Can you work these out from the model? Positions are in its coordinate system, mm. Face numbers are marked on the shaded views. A direction names the side the tool comes from. Coordinates: 2 decimals unless noted, no trailing zeros. Order: outer loops, then holes, each group sorted by start corner. A loop starts at its lowest first (then second) coordinate and runs counter-clockwise, first axis right, second up.
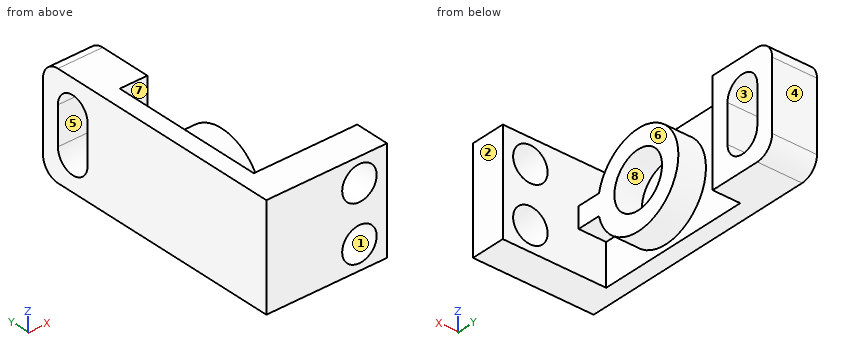
```python
from build123d import *

# Parameters (mm, degrees)
BASE_PLATE_SKETCH_W     = 35
BASE_PLATE_SKETCH_H     = 10
BASE_PLATE_DEPTH        = 30
UPRIGHT_WALL_SKETCH_W   = 5
UPRIGHT_WALL_SKETCH_H   = 45
UPRIGHT_WALL_DEPTH      = 30
MOUNTING_HOLES_SKETCH_R = 5
MOUNTING_HOLES_2X_DEPTH = 30
TOP_LUG_DEPTH           = 8
TOP_LUG_DEPTH_BACK      = 5
LUG_SLOT_DEPTH          = 84.719770664
RING_BOSS_SKETCH_R      = 8
RING_BOSS_DEPTH         = 8


with BuildPart() as part:
    # Base Plate Sketch → Base Plate (new body)
    with BuildSketch(Plane.XY):
        with Locations((17.5, 5)):
            Rectangle(BASE_PLATE_SKETCH_W, BASE_PLATE_SKETCH_H)
    extrude(amount=-BASE_PLATE_DEPTH)

    # Upright Wall Sketch → Upright Wall (add)
    with BuildSketch(Plane.XY):
        with Locations((2.5, 32.5)):
            Rectangle(UPRIGHT_WALL_SKETCH_W, UPRIGHT_WALL_SKETCH_H)
    extrude(amount=-UPRIGHT_WALL_DEPTH)

    # Mounting Holes Sketch → Mounting Holes 2x (cut)
    with BuildSketch(Plane(origin=(0, 10, 0), x_dir=(1, 0, 0), z_dir=(0, 1, 0))):
        with Locations(Location((27, 23, 0), (0, 0, 270))):
            Circle(MOUNTING_HOLES_SKETCH_R)
        with Locations(Location((27, 7, 0), (0, 0, 270))):
            Circle(MOUNTING_HOLES_SKETCH_R)
    extrude(amount=-MOUNTING_HOLES_2X_DEPTH, mode=Mode.SUBTRACT)

    # Top Lug Sketch → Top Lug (add, two sides: drawn at the far end of the back side and taken through both)
    with BuildSketch(Plane(origin=(5, 0, 0), x_dir=(0, 0, -1), z_dir=(1, 0, 0)).offset(-TOP_LUG_DEPTH_BACK)):
        with BuildLine():
            Line((0, 55), (30, 55))
            Line((30, 55), (30, 70))
            ThreePointArc((30, 70), (28.535533906, 73.535533906), (25, 75))
            Line((25, 75), (5, 75))
            ThreePointArc((5, 75), (1.464466094, 73.535533906), (0, 70))
            Line((0, 70), (0, 55))
        make_face()
    extrude(amount=TOP_LUG_DEPTH + TOP_LUG_DEPTH_BACK)

    # Lug Slot Sketch → Lug Slot (cut, through all)
    with BuildSketch(Plane(origin=(13, 0, 0), x_dir=(0, 0, -1), z_dir=(1, 0, 0))):
        with BuildLine():
            Line((9.5, 70), (20.5, 70))
            ThreePointArc((20.5, 70), (25.5, 65), (20.5, 60))
            Line((20.5, 60), (9.5, 60))
            ThreePointArc((9.5, 60), (4.5, 65), (9.5, 70))
        make_face()
    extrude(amount=-LUG_SLOT_DEPTH, mode=Mode.SUBTRACT)

    # Ring Boss Sketch → Ring Boss (add)
    with BuildSketch(Plane(origin=(5, 0, 0), x_dir=(0, 0, -1), z_dir=(1, 0, 0))):
        with BuildLine():
            Line((12, 16.837553419), (12, 10))
            Line((12, 10), (18, 10))
            Line((18, 10), (18, 16.837553419))
            ThreePointArc((18, 16.837553419), (15, 43.5), (12, 16.837553419))
        make_face()
        with Locations((15, 30)):
            Circle(RING_BOSS_SKETCH_R, mode=Mode.SUBTRACT)
    extrude(amount=RING_BOSS_DEPTH)


solid = part.part
```
1. Imagine slicing it at D-D on y = 12.5. Please give me the cut outline in (x, z), then the cut area to 3 significant figures.
Completed:
outline: (0, -30) - (5, -30) - (5, -18) - (13, -18) - (13, -12) - (5, -12) - (5, 0) - (0, 0) - close
area: 198 mm2
2. Thinking about a two-plate mould opening in X: for the marked faces 1, 2 and 3, which applies, pulls with the +X half, pulls with the -X half, needs draft (parallel to the pull), parting line crosses it, or undercut?
Completed:
face 1: undercut
face 2: pulls with the +X half
face 3: needs draft
3. Imagine slicing it at A-A on x = 12. Please give me the cut outline in (y, z).
Completed:
outline: (0, -30) - (10, -30) - (10, -18) - (16.84, -18) arc R13.5 ccw (long way) to (16.84, -12) - (10, -12) - (10, 0) - (0, 0) - close; (55, -30) - (70, -30) arc R5 ccw to (75, -25) - (75, -5) arc R5 ccw to (70, 0) - (55, 0) - close; hole circle Ø16 at (30, -15); hole (60, -20.5) arc R5 ccw to (70, -20.5) - (70, -9.5) arc R5 ccw to (60, -9.5) - close
4. I'm going to push flat-ended pins straight in: pin 1 (8 mm diameter, centred on y = 28.5, z = -17.5, fed in from +X); pin 2 (1 mm diameter, centred on x = 4, z = -3.5, fed in from +Y); pin 3 (3 mm diameter, centred on x = 7.5, y = 22, fed in from +Z). Where does each tip first touch, or does it pass through?
Completed:
pin 1: stops at x = 5
pin 2: stops at y = 74.9
pin 3: stops at z = -3.17
5. Imagine slicing it at B-B on z = -15. Please give me the cut outline in (x, y), then the cut area to 3 significant figures.
Completed:
outline: (0, 0) - (35, 0) - (35, 10) - (13, 10) - (13, 22) - (5, 22) - (5, 38) - (13, 38) - (13, 43.5) - (5, 43.5) - (5, 55) - (13, 55) - (13, 60) - (0, 60) - close; (0, 70) - (13, 70) - (13, 75) - (0, 75) - close
area: 845 mm2
6. On a 3-axis mill with a long thin cutter (end or side, diameter ignored), from which of +Z, -Z, +X, -X, +Y, -Y can I reach the whole of each face in a straight line? I mean the marked faces 4, 5, 6, 7 and 8. Say none if no direction works.
Completed:
face 4: +Z, -Z, +X, -X, +Y
face 5: +X, -X
face 6: +Z, -Z, +X, +Y
face 7: +Z, -Z, +X
face 8: +X
7. Please list where these lines run through material, in increasing order: probe 1 along Y at (x, z) = (7, -15); probe 2 along X at (y, z) = (5.5, -23); probe 3 along Y at (x, z) = (9, -5).
Completed:
probe 1: y = 0 to 22, 38 to 43.5, 55 to 60, 70 to 75
probe 2: x = 0 to 22, 32 to 35
probe 3: y = 0 to 10, 20.93 to 39.07, 55 to 62.82, 67.18 to 75
8. Imagine slicing it at C-C on x = 27. Please give me the cut outline in (y, z).
Completed:
outline: (0, -30) - (10, -30) - (10, -28) - (0, -28) - close; (0, -18) - (10, -18) - (10, -12) - (0, -12) - close; (0, -2) - (10, -2) - (10, 0) - (0, 0) - close
